Here's how the part is built. I have some questions about the finished solid (model axes, mm). Face numbers are marked on the shaded views. A direction names the side the tool comes from. Round coordinates to 2 decimals unless told otherwise and drop trailing zeros. Write each loop counter-clockwise with the first axis right and the second up, starting at its lowest first coordinate (ties: lowest second). Pieces come first, ordered by that corner, then holes. Notation, with made-up numbers: (61, 86.5) -> (89, 86.5) arc R17 ccw to (89, 105.5) -> close; hole circle Ø5 at (-1, -21.75). An arc over 180 degrees is marked (long way). Answer in a Markdown table with one row per item. Add a question column.
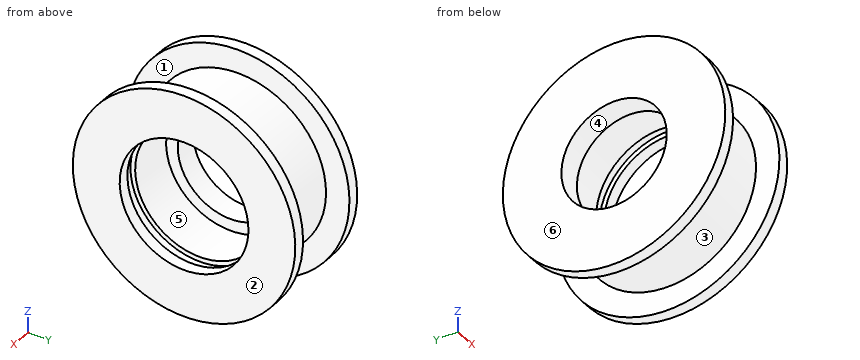
from build123d import *


with BuildPart() as part:
    # 草图1 → 旋转1 (revolve)
    with BuildSketch(Plane.XY, mode=Mode.PRIVATE) as revolve_1_sk:
        Polygon((-4, 4.5), (-2, 4.5), (-2, 5.5), (2, 5.5), (2, 5.9), (3, 5.9), (3, 5.5), (4, 5.5), (4, 9.5), (3, 9.5), (3, 7.5), (-3, 7.5), (-3, 9.5), (-4, 9.5), align=None)
    revolve(revolve_1_sk.sketch.rotate(Axis((4, 0, 0), (-1, 0, 0)), 270), axis=Axis((4, 0, 0), (-1, 0, 0)))


solid = part.part
Item 1: I need wall thicknesses on line 1 along X through (y, z) = (7.5, -1); line 2 along Y through (x, z) = (-3.1, 0); line 3 along Y through (x, z) = (2.7, 0). Which ranges of each line are inside material? Lowest first, please. Write a range as from..to.
Item 2: On a 3-axis mill with a long thin cutter (end or side, diameter ignored), from which of +Z, -Z, +X, -X, +Y, -Y can I reach the whole of each face in a straight line? I mean the marked faces 1 and 2. Say none if no direction works.
Item 3: If we mould it in two halves opening along Z, with no side actions, what happens to the marked faces 3, 4, 5 and 6? For each: pulls with the +Z half, pulls with the -Z half, needs draft (parallel to the pull), parting line crosses it, or undercut.
Item 4: If we section it at C-C on x = -1.5: Please give me the cut outline in (y, z), then the cut area to 3 significant figures.
Item 5: If we section it at D-D on y = -5: Please give me the cut outline in (x, z).
Item 6: If we section it at A-A on z = 0: Please give me the cut outline in (x, y), then the cut area to 3 significant figures.
Item 7: For P1, Ø5.5, axis at y = 0, z = 1, coming from the -X side; P2, Ø1.5, axis at x = -1.5, y = -1.5, coming from the -Z side; P3, Ø3, axis at x = -3, y = -4.5, coming from the +Z side; P4, Ø1.5, axis at x = 1.5, z = -4.5, coming from the -Y side, each with a flat end and sliding along its axis, tell me the tip position at first contact or that it passes through.
Results list:
| question | item | result |
|---|---|---|
| 1 | line 1 | -4..-3, 3..4 |
| 1 | line 2 | -9.5..-4.5, 4.5..9.5 |
| 1 | line 3 | -7.5..-5.9, 5.9..7.5 |
| 2 | face 1 | none |
| 2 | face 2 | +Z, -Z, +X, +Y, -Y |
| 3 | face 3 | parting line crosses it |
| 3 | face 4 | undercut |
| 3 | face 5 | undercut |
| 3 | face 6 | needs draft |
| 4 | outline | circle Ø15 at (0, 0); hole circle Ø11 at (0, 0) |
| 4 | area | 81.7 mm² |
| 5 | outline | (-4, -8.08) -> (-3, -8.08) -> (-3, -5.59) -> (3, -5.59) -> (3, -8.08) -> (4, -8.08) -> (4, -2.29) -> (3, -2.29) -> (3, -3.13) -> (2, -3.13) -> (2, -2.29) -> (-2, -2.29) -> (-2, 2.29) -> (2, 2.29) -> (2, 3.13) -> (3, 3.13) -> (3, 2.29) -> (4, 2.29) -> (4, 8.08) -> (3, 8.08) -> (3, 5.59) -> (-3, 5.59) -> (-3, 8.08) -> (-4, 8.08) -> close |
| 6 | outline | (-4, -9.5) -> (-3, -9.5) -> (-3, -7.5) -> (3, -7.5) -> (3, -9.5) -> (4, -9.5) -> (4, -5.5) -> (3, -5.5) -> (3, -5.9) -> (2, -5.9) -> (2, -5.5) -> (-2, -5.5) -> (-2, -4.5) -> (-4, -4.5) -> close; (-4, 4.5) -> (-2, 4.5) -> (-2, 5.5) -> (2, 5.5) -> (2, 5.9) -> (3, 5.9) -> (3, 5.5) -> (4, 5.5) -> (4, 9.5) -> (3, 9.5) -> (3, 7.5) -> (-3, 7.5) -> (-3, 9.5) -> (-4, 9.5) -> close |
| 6 | area | 43.2 mm² |
| 7 | P1 | through |
| 7 | P2 | z = -7.46 |
| 7 | P3 | z = 9.01 |
| 7 | P4 | y = -6.5 |
